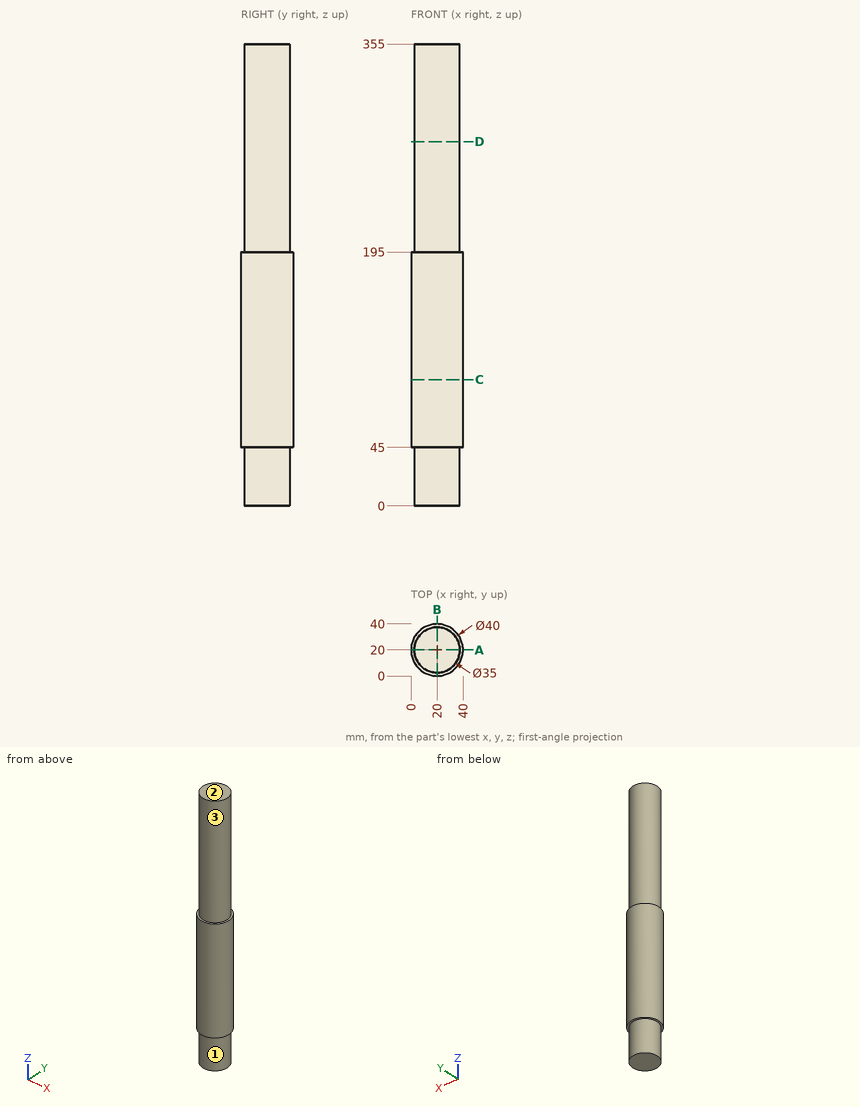
Study the drawing (mm; zero at the part's minimum x, y, z) and answer. A direction names the side the tool comes from. Round coordinates to 2 decimals unless told otherwise and drop trailing zeros. Write each loop counter-clockwise with the first axis right and the second up, starting at its lowest first coordinate (ties: lowest second). Pieces come first, ordered by that corner, then holes. Notation, with made-up numbers: (41, -39) -> (76, -39) arc R33 cw to (76, -4) -> close; hole circle Ø8 at (-24.5, 10). An arc over 180 degrees is marked (long way). Use CSV: the item, a comma, the result in double quotes. Start each with the question number.
(1) Section C-C on z = 97 is taken. Give the vertices of the cut face in (x, y).
(2) Section D-D on z = 280 is taken. Give the vertices of the cut face in (x, y).
(3) Consider L1, parallel to Y at x = 19.5, z = 57; L2, parallel to X at y = 18.5, z = 328; L3, parallel to Z at x = 21, y = 38.5. Determine where each line is inside the solid, lowest interval first. Write a range as from..to.
(4) Each of these flat-tipped pins is pushed along its axis until it touches: pin 1 (10 mm diameter, centred on x = 30.5, z = 197, fed in from +Y); pin 2 (1 mm diameter, centred on x = 35.5, z = 148, fed in from -Y); pin 3 (8 mm diameter, centred on x = 32.5, z = 272, fed in from -Y). Where does it stop, or does it pass through?
(5) Section A-A on y = 20 is taken. Give the vertices of the cut face in (x, z), then the cut area to 3 significant figures.
(6) Which of the six approach directions +Z, -Z, +X, -X, +Y, -Y give full straight-line access (tool end or side, diameter ignored) to the marked faces 1, 2 and 3?
A:
1,outline,"circle Ø40 at (20, 20)"
2,outline,"circle Ø35 at (20, 20)"
3,L1,"y = 0.01..39.99"
3,L2,"x = 2.56..37.44"
3,L3,"z = 45..195"
4,pin 1,"stops at y = 39.1"
4,pin 2,"stops at y = 6.77"
4,pin 3,"stops at y = 4.7"
5,outline,"(0, 45) -> (2.5, 45) -> (2.5, 0) -> (37.5, 0) -> (37.5, 45) -> (40, 45) -> (40, 195) -> (37.5, 195) -> (37.5, 355) -> (2.5, 355) -> (2.5, 195) -> (0, 195) -> close"
5,area,"13,200 mm²"
6,face 1,"-Z"
6,face 2,"+Z, +X, -X, +Y, -Y"
6,face 3,"+Z"
